```python
from build123d import *
from build123d.topology import SkipClean

# Parameters (mm, degrees)
LOWER_ARM_SKETCH_R  = 7.5
LOWER_ARM_DEPTH     = 6
HUB_BASE_SKETCH_R   = 13.5
HUB_BASE_BOSS_DEPTH = 9
PIVOT_BORE_SKETCH_R = 7.5
PIVOT_BORE_15_DEPTH = 96.291657557
END_BOSS_SKETCH_R   = 9.5
END_BOSS_SKETCH_R_2 = 5.5
END_BOSS_19_DEPTH   = 8.75
UPPER_ARM_DEPTH     = 6.25


with BuildPart() as part:
    # Lower Arm Sketch → Lower Arm (new, symmetric)
    with BuildSketch(Plane(origin=(0, 0, 0), x_dir=(1, 0, 0), z_dir=(0, 1, 0))):
        with BuildLine():
            Line((-45, 13.5), (0, 13.5))
            ThreePointArc((0, 13.5), (13.5, 0), (0, -13.5))
            Line((0, -13.5), (-45, -13.5))
            ThreePointArc((-45, -13.5), (-58.5, 0), (-45, 13.5))
        make_face()
        with Locations(Location((-45, 0, 0), (0, 0, 270))):
            Circle(LOWER_ARM_SKETCH_R, mode=Mode.SUBTRACT)
    extrude(amount=LOWER_ARM_DEPTH, both=True)

    # Hub Base Sketch → Hub Base Boss (add, symmetric)
    with SkipClean():  # the faces are left unmerged after this step: merging them gives an invalid solid
        with BuildSketch(Plane(origin=(0, 0, 0), x_dir=(1, 0, 0), z_dir=(0, 1, 0))):
            with Locations(Location((0, 0, 0), (0, 0, 270))):
                Circle(HUB_BASE_SKETCH_R)
        extrude(amount=HUB_BASE_BOSS_DEPTH, both=True)

    # Pivot Hub Profile → Pivot Hub (revolve)
    with SkipClean():  # the faces are left unmerged after this step: merging them gives an invalid solid
        with BuildSketch(Plane.XY, mode=Mode.PRIVATE) as pivot_hub_sk:
            Polygon((0, 0), (0, 65), (12.5, 65), (12.5, 62), (13.5, 62), (13.5, 44), (12.5, 44), (12.5, 0), align=None)
        revolve(pivot_hub_sk.sketch.rotate(Axis((0, 0, 0), (0, 1, 0)), 90), axis=Axis((0, 0, 0), (0, 1, 0)))

    # Pivot Bore Sketch → Pivot Bore Ø15 (cut, through all)
    with SkipClean():  # the faces are left unmerged after this step: merging them gives an invalid solid
        with BuildSketch(Plane(origin=(0, 65, 0), x_dir=(1, 0, 0), z_dir=(0, 1, 0))):
            with Locations(Location((0, 0, 0), (0, 0, 270))):
                Circle(PIVOT_BORE_SKETCH_R)
        extrude(amount=-PIVOT_BORE_15_DEPTH, mode=Mode.SUBTRACT)



with BuildPart() as body_2:
    # End Boss Sketch → End Boss Ø19 (new, symmetric)
    with BuildSketch(Plane(origin=(0, 53, 0), x_dir=(1, 0, 0), z_dir=(0, 1, 0))):
        with Locations(Location((0, -60, 0), (0, 0, 270))):
            Circle(END_BOSS_SKETCH_R)
        with Locations(Location((0, -60, 0), (0, 0, 270))):
            Circle(END_BOSS_SKETCH_R_2, mode=Mode.SUBTRACT)
    extrude(amount=END_BOSS_19_DEPTH, both=True)


with BuildPart() as part_1:
    with SkipClean():  # the faces are left unmerged after this step: merging them gives an invalid solid
        add(part.part)

        add(body_2.part)  # Upper Arm merges body 2
        # Upper Arm Sketch → Upper Arm (add, symmetric)
        with BuildSketch(Plane(origin=(0, 53, 0), x_dir=(1, 0, 0), z_dir=(0, 1, 0))):
            with BuildLine():
                Line((13.469966592, -0.9), (9.47886538, -60.633333333))
                ThreePointArc((9.47886538, -60.633333333), (0, -50.5), (-9.47886538, -60.633333333))
                Line((-9.47886538, -60.633333333), (-13.469966592, -0.9))
                ThreePointArc((-13.469966592, -0.9), (0, -13.5), (13.469966592, -0.9))
            make_face()
        extrude(amount=UPPER_ARM_DEPTH, both=True)


solid = part_1.part
```
Source: CAD feature listing. Evaluate the final solid. Frame: model axes, mm. A direction names the side the tool comes from. Coordinates: 2 decimals unless noted, no trailing zeros. Write each loop counter-clockwise with the first axis right and the second up, starting at its lowest first coordinate (ties: lowest second). Pieces come first, ordered by that corner, then holes. Notation, with made-up numbers: (49, 12.5) - (95, 12.5) arc R17 ccw to (95, 30.5) - close; hole circle Ø8 at (-20.75, 5.5). An arc over 180 degrees is marked (long way). Answer as a JSON object with one key per item and string values.
Q1. First-contact query: pin 1 Ø12 at (x, z) = (-45, 0) entering from +Y; pin 2 Ø5.5 at (x, z) = (2, 63) entering from -Y; pin 3 Ø5 at (x, y) = (-4.5, 46.5) entering from -Z; pin 4 Ø13.5 at (x, z) = (-43.5, 2.5) entering from +Y. Flat tips, straight axial feed; report the tip coordinate or a pass-through.
Ans:
{"pin 1": "passes through", "pin 2": "stops at y = 44.25", "pin 3": "stops at z = -13.35", "pin 4": "stops at y = 6"}
Q2. Material intervals for line 1 (X direction, y = 3.75, z = 0); line 2 (X direction, y = 58, z = 60); line 3 (X direction, y = 31, z = 0), sorted ascending. Write a range as [from, to].
Ans:
{"line 1": "x = [-58.5, -52.5], [-37.5, -7.5], [7.5, 13.5]", "line 2": "x = [-9.52, -5.5], [5.5, 9.52]", "line 3": "x = [-12.5, -7.5], [7.5, 12.5]"}
Q3. Section query C-C, the plane z = 46. Output: boundary loops of the cut face in (x, y), plus the area to 3 significant figures.
Ans:
{"outline": "(-10.46, 46.75) - (10.46, 46.75) - (10.46, 59.25) - (-10.46, 59.25) - close", "area": "261 mm2"}
Q4. Draft query along Z for faces 6 (the flat face through (11.502, 53.088, 30.349)), 7 (the flat face through (-29, 6, 0)), 8 (the cylindrical face through (0.33, 28.518, -7.493)). Return one class per face: released by +Z, released by -Z, zero draft, split by the parting line, or undercut.
Ans:
{"face 6": "released by +Z", "face 7": "zero draft", "face 8": "undercut"}
Q5. Section query B-B, the plane x = -30.5. Output: boundary loops of the cut face in (y, z).
Ans:
{"outline": "(-6, -13.5) - (6, -13.5) - (6, 13.5) - (-6, 13.5) - close"}
Q6. Section query A-A, the plane y = -3.5. Output: boundary loops of the cut face in (x, z), plus the area to 3 significant figures.
Ans:
{"outline": "(-45, -13.5) - (0, -13.5) arc R13.5 ccw to (0, 13.5) - (-45, 13.5) arc R13.5 ccw to start; hole circle Ø15 at (-45, 0); hole circle Ø15 at (0, 0)", "area": "1,430 mm2"}
Q7. Set-up query: faces 1 (the flat face through (-22, 0, 13.5)), 2 (the flat face through (9, 62, 9)), 3 (the flat face through (-4, 61.75, 64)), 4 (the cylindrical face through (-3.755, 26.255, -11.923)), 5 (the flat face through (-11.446, 53.088, 31.185)). Return all of +Z, -Z, +X, -X, +Y, -Y with unobstructed straight access to the full face (end or side cutting, diameter ignored); none if empty.
Ans:
{"face 1": "+Z, +X, -X, -Y", "face 2": "+Y", "face 3": "+Z, +X, -X, +Y", "face 4": "none", "face 5": "+Z, -X, +Y"}
